Print and shaded views of the part. All mm, measured from the part's lowest x, y and z. A direction names the side the tool comes from. Give positions to 0.01 mm unless a question says otherwise; leave off trailing zeros. Loops run counter-clockwise (first coordinate to the right, second up) from the corner with the lowest first, then second, coordinate; pieces in that order, holes last. Notation, with made-up numbers: M 35,-9.5 L 90,-9.5 A7 cw 90,-0.5 Z; hole C 24.25,-4 d6. An arc over 180 degrees is marked long. Answer in a Markdown table with one row per item.
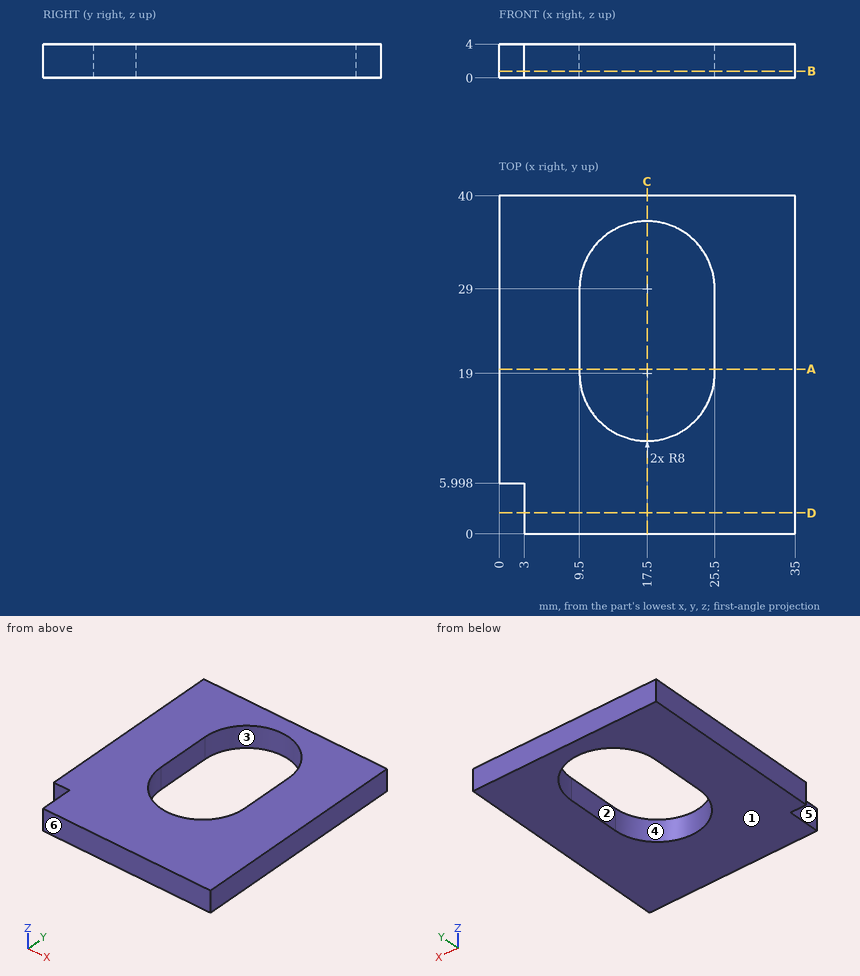
(1) Saw through at B-B, the plane z = 0.8. Give the cut face in (x, y).
Established:
| item | result |
|---|---|
| outline | M 0,6 L 3,6 L 3,0 L 35,0 L 35,40 L 0,40 Z; hole M 9.5,19 A8 ccw 25.5,19 L 25.5,29 A8 ccw 9.5,29 Z |
(2) Saw through at D-D, the plane y = 2.5. Give the cut face in (x, z).
Established:
| item | result |
|---|---|
| outline | M 3,0 L 35,0 L 35,4 L 3,4 Z |
(3) Saw through at C-C, the plane x = 17.5. Give the cut face in (y, z), and give its area (3 significant figures).
Established:
| item | result |
|---|---|
| outline | M 0,0 L 11,0 L 11,4 L 0,4 Z; M 37,0 L 40,0 L 40,4 L 37,4 Z |
| area | 56.0 mm2 |
(4) Flat gauge pins, fed straight in: P1, Ø2, axis at y = 3, z = 2.5, coming from the -X side; P2, Ø0.9, axis at x = 2, z = 1.5, coming from the -Y side; P3, Ø12, axis at x = 16.5, y = 24, coming from the -Z side. Where does each tip first touch, or does it go through?
Established:
| item | result |
|---|---|
| P1 | stops at x = 3 |
| P2 | stops at y = 6 |
| P3 | passes through |
(5) Wall check: L1, parallel to X at y = 25, z = 3.6; L2, parallel to X at y = 14.5, z = 1.65 (1 decimal); L3, parallel to X at y = 5.5, z = 2.4. Give the ranges that are in metal, low to high.
Established:
| item | result |
|---|---|
| L1 | x = 0 to 9.5, 25.5 to 35 |
| L2 | x = 0 to 10.9, 24.1 to 35 |
| L3 | x = 3 to 35 |
(6) Saw through at A-A, the plane y = 19.5. Give the cut face in (x, z), and give its area (3 significant figures).
Established:
| item | result |
|---|---|
| outline | M 0,0 L 9.5,0 L 9.5,4 L 0,4 Z; M 25.5,0 L 35,0 L 35,4 L 25.5,4 Z |
| area | 76.0 mm2 |
(7) Mould opens along X. For the marked faces 3, 4, 5 and 6 say: pulls with the +X half, pulls with the -X half, needs draft (parallel to the pull), parting line crosses it, or undercut.
Established:
| item | result |
|---|---|
| face 3 | undercut |
| face 4 | undercut |
| face 5 | pulls with the -X half |
| face 6 | needs draft |
(8) Which spindle directions (+Z, -Z, +X, -X, +Y, -Y) get a long thin tool onto all of the face, cutting with end or side? Do the marked faces 1 and 2. Say none if no direction does.
Established:
| item | result |
|---|---|
| face 1 | -Z, +X, -X, +Y, -Y |
| face 2 | +Z, -Z |
